Geometry check sheet. Reference: drawing and pictorial views, mm from the part's lowest x, y, z. A direction names the side the tool comes from. Coordinates: 2 decimals unless noted, no trailing zeros. Loops run counter-clockwise (first coordinate to the right, second up) from the corner with the lowest first, then second, coordinate; pieces in that order, holes last. Notation, with made-up numbers: (21.5, 85.5) - (68.5, 85.5) arc R29 ccw to (68.5, 110.5) - close; hole circle Ø8 at (0.5, -10). An arc over 180 degrees is marked (long way). One line per item, written item: value.
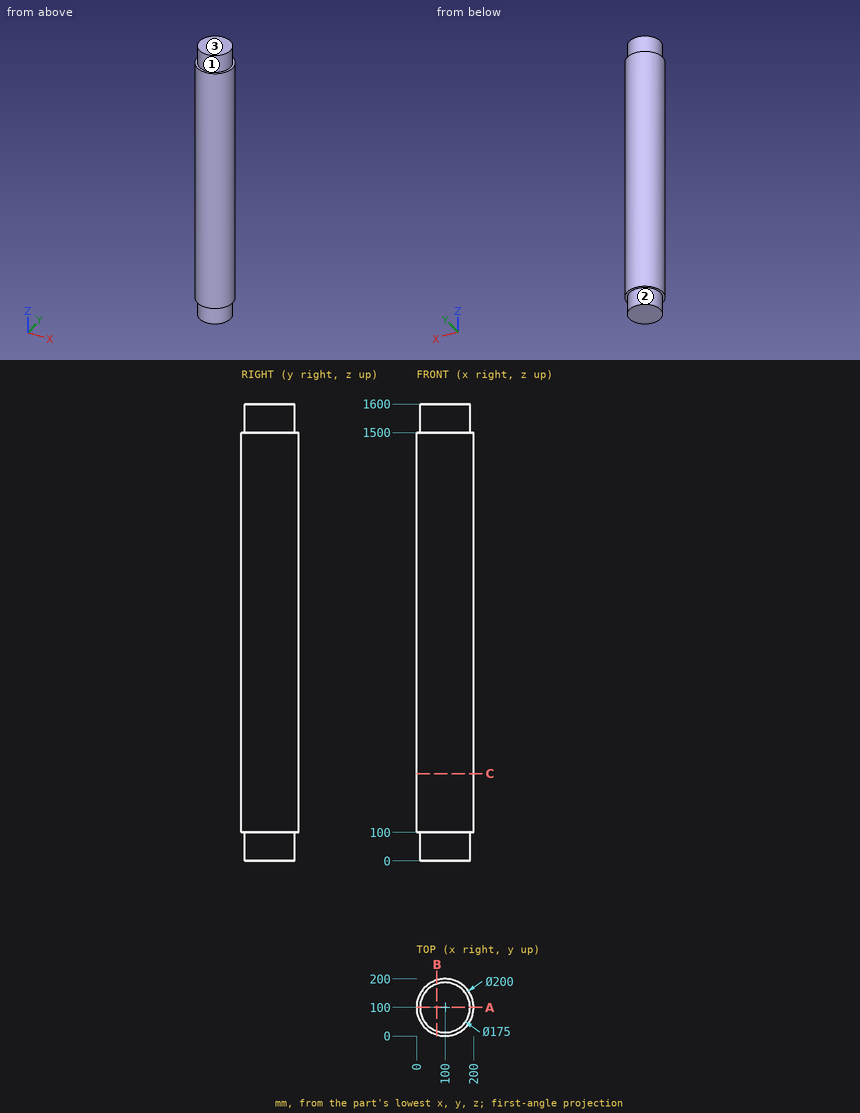
(1) Access from +Z, -Z, +X, -X, +Y, -Y to the whole of each face (thin tool, end or side, straight path). Record for the marked faces 1, 2 and 3.
Reply:
face 1: +Z
face 2: -Z
face 3: +Z, +X, -X, +Y, -Y
(2) Go/stop test with flat-tipped pins: pin 1 Ø3 at (y, z) = (98, 1081.5) entering from -X; pin 2 Ø4 at (y, z) = (144.5, 1208) entering from +X; pin 3 Ø6 at (x, y) = (22.5, 114) entering from -Z; pin 4 Ø2 at (x, z) = (88.5, 852.5) entering from -Y. Record where each tip stops, or that it passes through.
Reply:
pin 1: x = 0
pin 2: x = 190.52
pin 3: z = 0
pin 4: y = 0.55
(3) Cross-section at C-C on z = 305.5. Record the cut outline in (x, y), and give its area (3 significant figures).
Reply:
outline: circle Ø200 at (100, 100)
area: 31,400 mm2
(4) Material ranges on probe 1 along X at (y, z) = (96, 1507); probe 2 along X at (y, z) = (100.5, 773.5); probe 3 along Z at (x, y) = (184.5, 61), recorded low to high. Write a range as from..to.
Reply:
probe 1: 12.59..187.41
probe 2: 0..200
probe 3: 100..1500
(5) Cross-section at A-A on y = 100. Record the cut outline in (x, z).
Reply:
outline: (0, 100) - (12.5, 100) - (12.5, 0) - (187.5, 0) - (187.5, 100) - (200, 100) - (200, 1500) - (187.5, 1500) - (187.5, 1600) - (12.5, 1600) - (12.5, 1500) - (0, 1500) - close
(6) Cross-section at B-B on x = 71. Record the cut outline in (y, z), and give its area (3 significant figures).
Reply:
outline: (4.3, 100) - (17.45, 100) - (17.45, 0) - (182.55, 0) - (182.55, 100) - (195.7, 100) - (195.7, 1500) - (182.55, 1500) - (182.55, 1600) - (17.45, 1600) - (17.45, 1500) - (4.3, 1500) - close
area: 301,000 mm2
